Answer from the drawing. Dimensions are ordinates in mm from the lowest x, y and z of the part. Give positions to 0.01 mm unless a question says otherwise; leave off trailing zeros. Write each loop counter-clockwise with the first axis right and the second up, starting at its lowest first coordinate (ties: lowest second). Pieces come first, ordered by that corner, then holes. Notation, with made-up numbers: M 78.25,30 L 84.25,30 A15 ccw 84.25,49 Z; hole C -28.75,9 d1. An arc over 180 degrees is marked long. Answer as a JSON object with one key per item and string values.
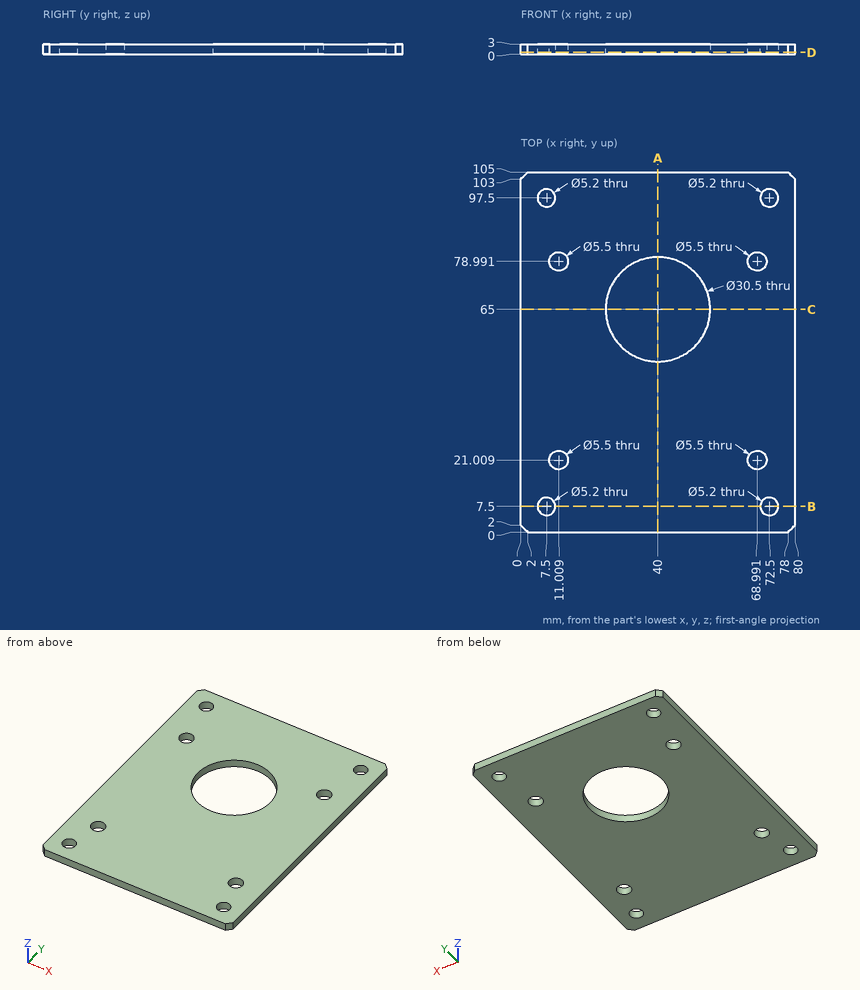
1. Flat-ended cylindrical pins translate along their axes: pin 1 (3.5 mm diameter, centred on x = 68.99, y = 21.01, fed in from -Z); pin 2 (6.5 mm diameter, centred on x = 68.99, y = 78.99, fed in from +Z). Find the tip coordinate at first contact, or state that the pin passes through.
Verdict:
{"pin 1": "passes through", "pin 2": "stops at z = 3"}
2. Consider line 1 along Y through (x, z) = (7.5, 1.1); line 2 along Y through (x, z) = (74.5, 0.5); line 3 along X through (y, z) = (22.5, 1.55). Determine where each line is inside the solid, lowest interval first.
Verdict:
{"line 1": "y = 0 to 4.9, 10.1 to 94.9, 100.1 to 105", "line 2": "y = 0 to 5.84, 9.16 to 95.84, 99.16 to 105", "line 3": "x = 0 to 8.7, 13.32 to 66.68, 71.3 to 80"}
3. A cutting plane is placed at D-D, the plane z = 0.55. Count the separate pieces of the cut face and the enclosed holes in it, plus the area to 3 significant figures.
Verdict:
{"separate pieces": "1", "enclosed holes": "9", "area": "7,480 mm2"}
4. A cutting plane is placed at B-B, the plane y = 7.5. Give the vertices of the cut face in (x, z).
Verdict:
{"outline": "M 0,0 L 4.9,0 L 4.9,3 L 0,3 Z; M 10.1,0 L 69.9,0 L 69.9,3 L 10.1,3 Z; M 75.1,0 L 80,0 L 80,3 L 75.1,3 Z"}
5. A cutting plane is placed at C-C, the plane y = 65. Give the vertices of the cut face in (x, z).
Verdict:
{"outline": "M 0,0 L 24.75,0 L 24.75,3 L 0,3 Z; M 55.25,0 L 80,0 L 80,3 L 55.25,3 Z"}
6. A cutting plane is placed at A-A, the plane x = 40. Give the vertices of the cut face in (y, z).
Verdict:
{"outline": "M 0,0 L 49.75,0 L 49.75,3 L 0,3 Z; M 80.25,0 L 105,0 L 105,3 L 80.25,3 Z"}
